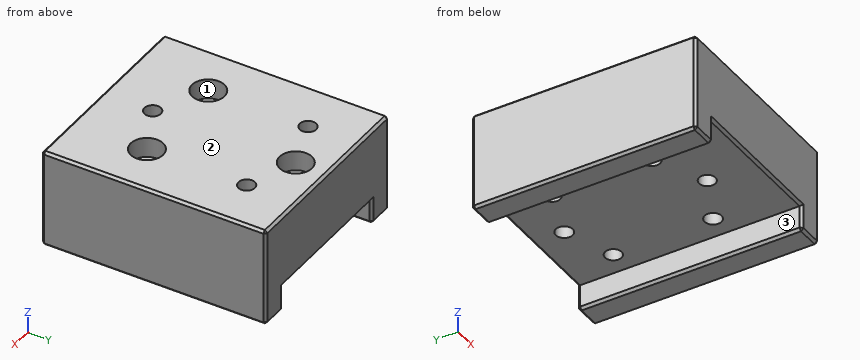
from build123d import *

# Parameters (mm, degrees)
SKETCH_1_W                   = 40
SKETCH_1_H                   = 45
EXTRUDE_1_DEPTH              = 7.35
HOLE_WIZARD_M3_1_D           = 3.4
HOLE_WIZARD_M3_1_CBORE_D     = 6.5
HOLE_WIZARD_M3_1_CBORE_DEPTH = 4
SKETCH_5_W                   = 5.4
SKETCH_5_H                   = 45
EXTRUDE_2_DEPTH              = 5
HOLE_WIZARD_M4_2_D           = 3.3
CHAMFER_1_SIZE               = 0.5


with BuildPart() as part:
    # 草图1 → 凸台-拉伸1 (new, symmetric)
    with BuildSketch(Plane.XY):
        Rectangle(SKETCH_1_W, SKETCH_1_H)
    extrude(amount=EXTRUDE_1_DEPTH, both=True)

    # M3 六角凹头螺钉的柱形沉头孔1 (through all)
    with Locations(Plane.XY.offset(7.35)):
        with Locations((0, 16.2), (-10, -7.5), (10, -7.5)):
            CounterBoreHole(HOLE_WIZARD_M3_1_D / 2, HOLE_WIZARD_M3_1_CBORE_D / 2, HOLE_WIZARD_M3_1_CBORE_DEPTH)

    # 草图5 → 凸台-拉伸2 (add)
    with BuildSketch(Plane(origin=(0, 0, -7.35), x_dir=(-1, 0, 0), z_dir=(0, 0, -1))):
        with Locations((-17.3, 0)):
            Rectangle(SKETCH_5_W, SKETCH_5_H)
        with Locations((17.3, 0)):
            Rectangle(SKETCH_5_W, SKETCH_5_H)
    extrude(amount=EXTRUDE_2_DEPTH)

    # M4 螺纹孔2 (through all)
    with Locations(Plane.XY.offset(7.35)):
        with Locations((10, 12.5), (-10, 12.5), (0, -12.5)):
            Hole(HOLE_WIZARD_M4_2_D / 2)

    # 倒角1
    chamfer_1_edges = [part.edges().sort_by_distance(p)[0] for p in [
        (-20, 0, 7.35),
        (0, -22.5, 7.35),
        (0, 22.5, -7.35),
        (14.6, -22.5, -9.85),
        (14.6, 22.5, -9.85),
        (20, 0, -12.35),
        (17.3, -22.5, -12.35),
        (14.6, 0, -12.35),
        (17.3, 22.5, -12.35),
        (20, 0, 7.35),
        (0, -22.5, -7.35),
        (-14.6, 22.5, -9.85),
        (-14.6, -22.5, -9.85),
        (-14.6, 0, -12.35),
        (-17.3, -22.5, -12.35),
        (-20, 0, -12.35),
        (-17.3, 22.5, -12.35),
        (0, 22.5, 7.35),
        (20, -22.5, -2.5),
        (-20, -22.5, -2.5),
        (-20, 22.5, -2.5),
        (20, 22.5, -2.5),
    ]]
    chamfer(chamfer_1_edges, length=CHAMFER_1_SIZE)


solid = part.part
Could you check a few things on this model? Use its own coordinates, in mm. Face numbers are marked on the shaded views. A direction names the side the tool comes from. Give positions to 0.01 mm unless a question says otherwise; leave off trailing zeros. Order: outer loops, then holes, each group sorted by start corner. A loop starts at its lowest first (then second) coordinate and runs counter-clockwise, first axis right, second up. Notation, with made-up numbers: (55, 29.25) - (71, 29.25) arc R22 cw to (71, 57.25) - close; hole circle Ø3 at (21, 33). An arc over 180 degrees is marked (long way). One line per question, with ' | ' between items. Start each with the question number.
Item 1: I want a section at D-D on y = -15. Write out the boundary of the cut face in (x, z).
Item 2: I want a section at C-C on x = 0. Write out the boundary of the cut face in (y, z), then the cut area to 3 significant figures.
Item 3: I need wall thicknesses on probe 1 along Y at (x, z) = (0, -2.5); probe 2 along Y at (x, z) = (-10, 5.75); probe 3 along X at (y, z) = (-14.5, -7.5). Which ranges of each line are inside material? Lowest first, please. Write a range as [from, to].
Item 4: I want a section at B-B on z = -1.25. Write out the boundary of the cut face in (x, y), then the cut area to 3 significant figures.
Item 5: For the marked faces 1, 2 and 3, which set-ups out of +Z, -Z, +X, -X, +Y, -Y let a thin tool reach every point of the face, with its end or its side?
Item 6: I want a section at A-A on y = 16.2. Write out the boundary of the cut face in (x, z), then the cut area to 3 significant figures.
Item 7: I'm going to push flat-ended pins straight in: pin 1 Ø6 at (x, y) = (-10, -7.5) entering from -Z; pin 2 Ø3 at (x, y) = (-13.5, -5) entering from -Z; pin 3 Ø2 at (x, y) = (0.5, 15.5) entering from +Z. Where does each tip first touch, or does it pass through?
Verdict:
1) outline: (-20, -11.85) - (-19.5, -12.35) - (-15.1, -12.35) - (-14.6, -11.85) - (-14.6, -7.35) - (14.6, -7.35) - (14.6, -11.85) - (15.1, -12.35) - (19.5, -12.35) - (20, -11.85) - (20, 6.85) - (19.5, 7.35) - (-19.5, 7.35) - (-20, 6.85) - close
2) outline: (-22.5, -6.85) - (-22, -7.35) - (-14.15, -7.35) - (-14.15, 7.35) - (-22, 7.35) - (-22.5, 6.85) - close; (-10.85, -7.35) - (14.5, -7.35) - (14.5, 3.35) - (12.95, 3.35) - (12.95, 7.35) - (-10.85, 7.35) - close; (17.9, -7.35) - (22, -7.35) - (22.5, -6.85) - (22.5, 6.85) - (22, 7.35) - (19.45, 7.35) - (19.45, 3.35) - (17.9, 3.35) - close | area: 550 mm^2
3) probe 1: [-22.5, -14.15], [-10.85, 14.5], [17.9, 22.5] | probe 2: [-22.5, -10.75], [-4.25, 10.85], [14.15, 22.5] | probe 3: [-20, -14.6], [14.6, 20]
4) outline: (-20, -22) - (-19.5, -22.5) - (19.5, -22.5) - (20, -22) - (20, 22) - (19.5, 22.5) - (-19.5, 22.5) - (-20, 22) - close; hole circle Ø3.4 at (-10, -7.5); hole circle Ø3.3 at (-10, 12.5); hole circle Ø3.4 at (0, 16.2); hole circle Ø3.3 at (0, -12.5); hole circle Ø3.4 at (10, -7.5); hole circle Ø3.3 at (10, 12.5) | area: 1,750 mm^2
5) face 1: +Z | face 2: +Z, +X, -X, +Y, -Y | face 3: -Z, +Y, -Y
6) outline: (-20, -11.85) - (-19.5, -12.35) - (-15.1, -12.35) - (-14.6, -11.85) - (-14.6, -7.35) - (-1.7, -7.35) - (-1.7, 3.35) - (-3.25, 3.35) - (-3.25, 7.35) - (-19.5, 7.35) - (-20, 6.85) - close; (1.7, -7.35) - (14.6, -7.35) - (14.6, -11.85) - (15.1, -12.35) - (19.5, -12.35) - (20, -11.85) - (20, 6.85) - (19.5, 7.35) - (3.25, 7.35) - (3.25, 3.35) - (1.7, 3.35) - close | area: 579 mm^2
7) pin 1: z = -7.35 | pin 2: z = -12.25 | pin 3: z = 3.35
